Could you check a few things on this drawing? It's one solid part, dimensions in mm from its lowest x, y, z. Give positions to 0.01 mm unless a question says otherwise; leave off trailing zeros. Order: outer loops, then holes, each group sorted by start corner. A loop starts at its lowest first (then second) coordinate and runs counter-clockwise, first axis right, second up.
(1) Imagine slicing it at A-A, the plane x = 38.1. Write out the boundary of the cut face in (y, z), then the cut area to 3 significant figures.
(2) Will this pin go through, and if not, where does the flat tip stop? pin 1 (16.5 mm diameter, centred on x = 38.1, y = 25.4, fed in from +Z).
(3) Imagine slicing it at C-C, the plane z = 6.5. Write out the boundary of the cut face in (x, y) (1 decimal).
(4) Imagine slicing it at B-B, the plane y = 25.4. Write out the boundary of the cut face in (x, z).
(5) If we mould it in two halves opening along X, with no side actions, what happens to the marked faces 1, 2 and 3? For each: released by +X, released by -X, zero draft, split by the parting line, or undercut.
(6) If I drill on probe 1 along Y at (x, z) = (38.1, 4), over which ranges is the centre line in solid material (lowest first)?
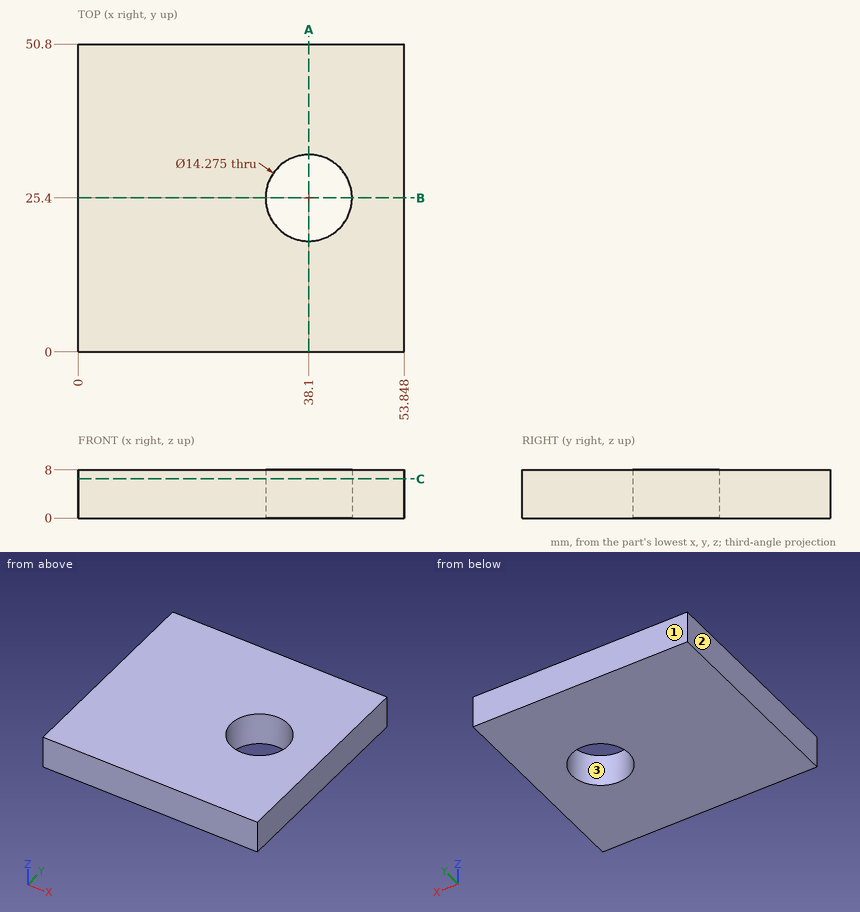
Answer block:
1. outline: (0, 0) - (18.26, 0) - (18.26, 8) - (0, 8) - close; (32.54, 0) - (50.8, 0) - (50.8, 8) - (32.54, 8) - close
1. area: 292 mm2
2. pin 1: stops at z = 8
3. outline: (0, 0) - (53.8, 0) - (53.8, 50.8) - (0, 50.8) - close; hole circle Ø14.3 at (38.1, 25.4)
4. outline: (0, 0) - (30.96, 0) - (30.96, 8) - (0, 8) - close; (45.24, 0) - (53.85, 0) - (53.85, 8) - (45.24, 8) - close
5. face 1: zero draft
5. face 2: released by -X
5. face 3: undercut
6. probe 1: y = 0 to 18.26, 32.54 to 50.8
